Read the model definition and answer for the solid it produces. Units are mm, in the model's axes. A direction names the side the tool comes from. Coordinates: 2 decimals unless noted, no trailing zeros. Order: outer loops, then holes, each group sorted by start corner. A loop starts at its lowest first (then second) coordinate and runs counter-clockwise, first axis right, second up. Notation, with made-up numbers: M 17,59.5 L 71,59.5 A24 ccw 71,72.5 Z; hole C -3,18.5 d7. An arc over 180 degrees is marked long. Use a Markdown table: item, result. Add a question column.
1) Find the intervals of material crossed by probe 1 along Y at (x, z) = (0, 65); probe 2 along Y at (x, z) = (0, 23); probe 3 along Z at (x, y) = (-32.5, -30), in increasing order. Write a range as [from, to].
2) Find section A-A on x = 0. Write down the section's boundary in (y, z), plus the area to 3 significant figures.
3) Each of these flat-tipped pins is pushed along its axis until it touches: pin 1 Ø12 at (y, z) = (-12.5, 26) entering from -X; pin 2 Ø5 at (x, y) = (22, 28.5) entering from -Z; pin 3 Ø6 at (x, z) = (28.5, 69.5) entering from +Y; pin 4 Ø4 at (y, z) = (-20.5, 61.5) entering from -X. Where does it stop, or does it pass through?
4) The mould has two halves that part along X. Classify faces 1 (the face through (-32.4, -5.7, 95)), 2 (the face through (37.815, 11.908, 94.854)), 3 (the face through (31, 9.76, 46.84)): released by +X, released by -X, zero draft, split by the parting line, or undercut.
5) Find section C-C on z = 33.5. Write down the section's boundary in (x, y), plus the area to 3 significant figures.
6) For faces 4 (the face through (23, -36, 30)), 5 (the face through (3, -33, 0)), determine the directions among +Z, -Z, +X, -X, +Y, -Y from which every point of the face is accessible in a straight line to the end or side of a thin tool.
from build123d import *

# Parameters (mm, degrees)
SKETCH_1_R          = 44.5
SKETCH_1_R_2        = 32.5
EXTRUDE_1_DEPTH     = 95
CUT_EXTRUDE_START   = -65
SKETCH_2_R          = 44.5
SKETCH_2_R_2        = 42.5
CUT_EXTRUDE_1_DEPTH = 65
CHAMFER_1_SIZE      = 3


with BuildPart() as part:
    # 草图1 → 凸台-拉伸1 (new body)
    with BuildSketch(Plane.XY):
        Circle(SKETCH_1_R)
        Circle(SKETCH_1_R_2, mode=Mode.SUBTRACT)
    extrude(amount=EXTRUDE_1_DEPTH)

    # 草图2 → 切除-拉伸1 (cut)
    with BuildSketch(Plane.XY.offset(95).offset(CUT_EXTRUDE_START)):
        Circle(SKETCH_2_R)
        Circle(SKETCH_2_R_2, mode=Mode.SUBTRACT)
    extrude(amount=CUT_EXTRUDE_1_DEPTH, mode=Mode.SUBTRACT)

    # 倒角1
    chamfer_1_edges = [part.edges().sort_by_distance(p)[0] for p in [
        (-42.5, 0, 95),
    ]]
    chamfer(chamfer_1_edges, length=CHAMFER_1_SIZE)


solid = part.part
Check result:
| question | item | result |
|---|---|---|
| 1 | probe 1 | y = [-42.5, -32.5], [32.5, 42.5] |
| 1 | probe 2 | y = [-44.5, -32.5], [32.5, 44.5] |
| 1 | probe 3 | z = [0, 30] |
| 2 | outline | M -44.5,0 L -32.5,0 L -32.5,95 L -39.5,95 L -42.5,92 L -42.5,30 L -44.5,30 Z; M 32.5,0 L 44.5,0 L 44.5,30 L 42.5,30 L 42.5,92 L 39.5,95 L 32.5,95 Z |
| 2 | area | 2,010 mm2 |
| 3 | pin 1 | stops at x = -44.02 |
| 3 | pin 2 | stops at z = 0 |
| 3 | pin 3 | stops at y = 34 |
| 3 | pin 4 | stops at x = -38.26 |
| 4 | face 1 | zero draft |
| 4 | face 2 | split by the parting line |
| 4 | face 3 | undercut |
| 5 | outline | C 0,0 d85; hole C 0,0 d65 |
| 5 | area | 2,360 mm2 |
| 6 | face 4 | +Z |
| 6 | face 5 | -Z, +X, -X, +Y, -Y |
